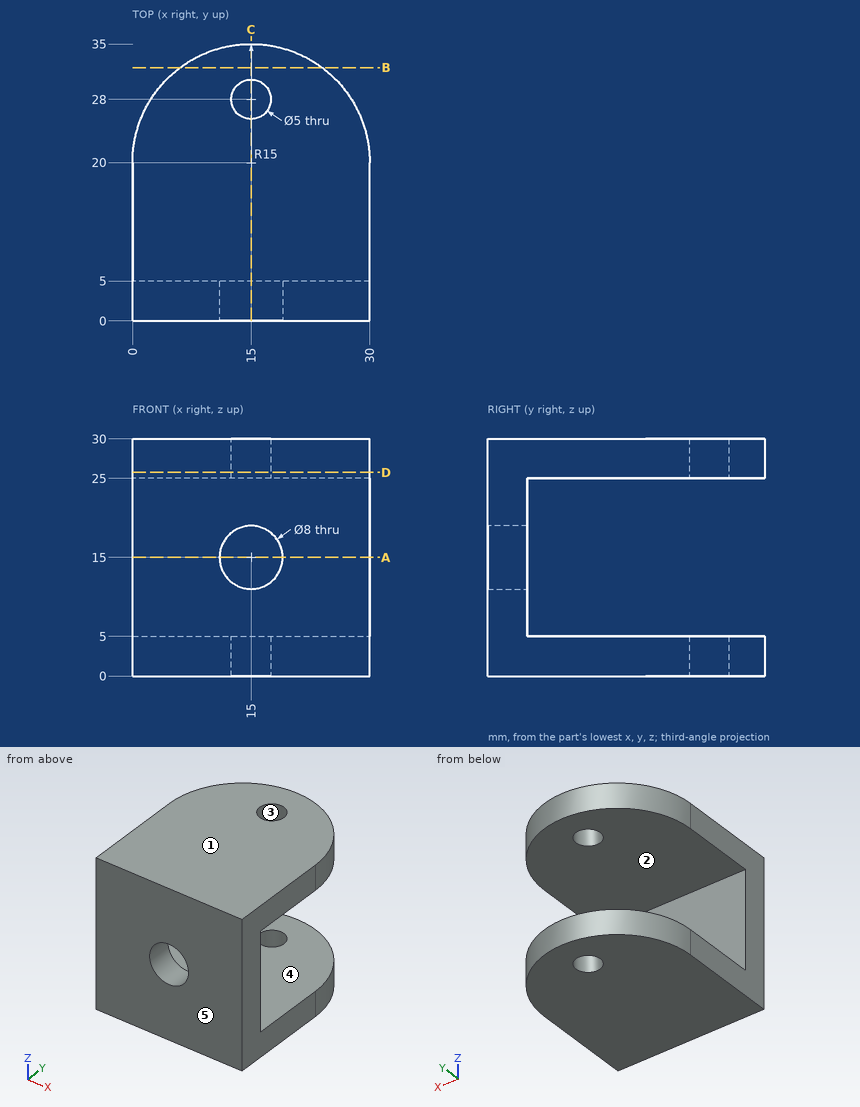
The drawing under review shows one solid part. Ordinate dimensions are in mm from its lowest x, y, z. A direction names the side the tool comes from. Coordinates: 2 decimals unless noted, no trailing zeros. Loops run counter-clockwise (first coordinate to the right, second up) from the corner with the lowest first, then second, coordinate; pieces in that order, holes last.
Item 1: Add section A-A (z = 15). Write out the cut boundary in (x, y).
Completed:
outline: (0, 0) - (11, 0) - (11, 5) - (0, 5) - close; (19, 0) - (30, 0) - (30, 5) - (19, 5) - close
Item 2: Wall thickness on L1, parallel to Z at x = 25.5, y = 22; L2, parallel to Y at x = 15, z = 28.3; L3, parallel to Y at x = 9.25, z = 5.5: over which ranges is each line inside the solid? List them lowest first.
Completed:
L1: z = 0 to 5, 25 to 30
L2: y = 0 to 25.5, 30.5 to 35
L3: y = 0 to 5
Item 3: Draft analysis for pull direction Y (two halves, no side actions). For the marked faces 3, 4 and 5, state which applies: pulls with the +Y half, pulls with the -Y half, needs draft (parallel to the pull), parting line crosses it, or undercut.
Completed:
face 3: undercut
face 4: needs draft
face 5: pulls with the -Y half
Item 4: Add section D-D (z = 25.75). Write out the cut boundary in (x, y).
Completed:
outline: (0, 0) - (30, 0) - (30, 20) arc R15 ccw to (0, 20) - close; hole circle Ø5 at (15, 28)
Item 5: For the marked faces 1 and 2, list the 3-axis set-ups (+Z, -Z, +X, -X, +Y, -Y) from which the entire face can be reached by the end or side of a thin tool; tool diameter is ignored.
Completed:
face 1: +Z, +X, -X, +Y, -Y
face 2: +X, -X, +Y
Item 6: Add section B-B (y = 32). Write out the cut boundary in (x, z), and give its area (3 significant figures).
Completed:
outline: (6, 0) - (24, 0) - (24, 5) - (6, 5) - close; (6, 25) - (24, 25) - (24, 30) - (6, 30) - close
area: 180 mm2
Item 7: Clearance check with flat-ended pins moving along their axes: pin 1 (10 mm diameter, centred on x = 9, z = 19, fed in from +Y); pin 2 (3 mm diameter, centred on x = 26.5, z = 25.5, fed in from +Y); pin 3 (10 mm diameter, centred on x = 21.5, z = 22.5, fed in from +Y). State where each tip first meets the part, or that it passes through.
Completed:
pin 1: stops at y = 5
pin 2: stops at y = 31.18
pin 3: stops at y = 34.84
Item 8: Add section C-C (x = 15). Write out the cut boundary in (y, z), and give its area (3 significant figures).
Completed:
outline: (0, 0) - (25.5, 0) - (25.5, 5) - (5, 5) - (5, 11) - (0, 11) - close; (0, 19) - (5, 19) - (5, 25) - (25.5, 25) - (25.5, 30) - (0, 30) - close; (30.5, 0) - (35, 0) - (35, 5) - (30.5, 5) - close; (30.5, 25) - (35, 25) - (35, 30) - (30.5, 30) - close
area: 360 mm2
